```python
from build123d import *

# Parameters (mm, degrees)
SLOTTED_BASE_PLATE_DEPTH = 14
REAR_UPRIGHT_BLOCK_DEPTH = 23
UPPER_STEP_BLOCK_DEPTH   = 9
TOP_BLOCK_DEPTH          = 9


with BuildPart() as part:
    # Slotted Base Plate Sketch → Slotted Base Plate (new body)
    with BuildSketch(Plane(origin=(0, 0, 0), x_dir=(1, 0, 0), z_dir=(0, 1, 0))):
        Polygon((-45.527413465, -5.526673775), (-45.527413465, -13.526673775), (-36.527413465, -13.526673775), (-36.527413465, 32.473326225), (-45.527413465, 32.473326225), (-45.527413465, 24.473326225), (-54.527413465, 24.473326225), (-54.527413465, -5.526673775), align=None)
        with BuildLine():
            ThreePointArc((5.472586535, 16.473326225), (-1.527413465, 9.473326225), (5.472586535, 2.473326225))
            Line((5.472586535, 2.473326225), (27.472586535, 2.473326225))
            Line((27.472586535, 2.473326225), (27.472586535, -8.526673775))
            Line((27.472586535, -8.526673775), (-10.527413465, -13.526673775))
            Line((-10.527413465, -13.526673775), (-36.527413465, -13.526673775))
            Line((-36.527413465, -13.526673775), (-36.527413465, 32.473326225))
            Line((-36.527413465, 32.473326225), (-10.527413465, 32.473326225))
            Line((-10.527413465, 32.473326225), (27.472586535, 27.473326225))
            Line((27.472586535, 27.473326225), (27.472586535, 16.473326225))
            Line((27.472586535, 16.473326225), (5.472586535, 16.473326225))
        make_face()
    extrude(amount=SLOTTED_BASE_PLATE_DEPTH)

    # Rear Upright Block Sketch → Rear Upright Block (add)
    with BuildSketch(Plane(origin=(0, 0, 0), x_dir=(1, 0, 0), z_dir=(0, 1, 0))):
        Polygon((-45.527413465, 32.473326225), (-36.527413465, 32.473326225), (-36.527413465, -13.526673775), (-45.527413465, -13.526673775), (-45.527413465, -5.526673775), (-54.527413465, -5.526673775), (-54.527413465, 24.473326225), (-45.527413465, 24.473326225), align=None)
    extrude(amount=REAR_UPRIGHT_BLOCK_DEPTH)

    # Upper Step Sketch → Upper Step Block (add)
    with BuildSketch(Plane(origin=(-36.527413465, 0, 0), x_dir=(0, 0, -1), z_dir=(1, 0, 0))):
        Polygon((-13.526673775, 23), (32.473326225, 23), (16.473326225, 32.368724422), (2.473326225, 32.368724422), align=None)
    extrude(amount=-UPPER_STEP_BLOCK_DEPTH)

    # Top Block Sketch → Top Block (add)
    with BuildSketch(Plane.ZY.offset(45.527413465)):
        Polygon((-24.473326225, 23), (-24.473326225, 27.684362211), (-16.473326225, 32.368724422), (-2.473326225, 32.368724422), (5.526673775, 27.684362211), (5.526673775, 23), align=None)
    extrude(amount=TOP_BLOCK_DEPTH)


solid = part.part
```
The listing builds one solid part. Answer for the finished solid, in the listing's coordinates (mm). A direction names the side the tool comes from. Give positions to 0.01 mm unless a question says otherwise; leave off trailing zeros. Order: outer loops, then holes, each group sorted by start corner. A loop starts at its lowest first (then second) coordinate and runs counter-clockwise, first axis right, second up. Notation, with made-up numbers: M 72.5,-14 L 77.5,-14 A12 ccw 77.5,0 Z; hole C 82,12 d3. An arc over 180 degrees is marked long. Put each result on its own line as item: value. Start each with the question number.
Item 1: The part is cut by section D-D, the plane y = 19.5. Determine the outline of the cut face in (x, z).
Item 2: The part is cut by section B-B, the plane x = 8. Determine the outline of the cut face in (y, z).
Item 3: The part is cut by section A-A, the plane y = 10. Determine the outline of the cut face in (x, z), and give its area (3 significant figures).
Item 4: The part is cut by section C-C, the plane z = -22.5. Determine the outline of the cut face in (x, y), and give its area (3 significant figures).
Item 5: Flat-ended cylindrical pins translate along their axes: P1, Ø2.5, axis at y = 16.5, z = 10.5, coming from the -X side; P2, Ø4, axis at x = 13.5, y = 6.5, coming from the +Z side; P3, Ø9, axis at y = 20, z = -27.5, coming from the -X side; P4, Ø7, axis at x = -51, y = 11.5, coming from the -Z side. Find the tip coordinate at first contact, or state that the pin passes through.
Item 6: Which of the six approach directions +Z, -Z, +X, -X, +Y, -Y give full straight-line access (tool end or side, diameter ignored) to faces 5 (the face through (-12, 14, -10)), 6 (the face through (-50, 14, -24.473)), 7 (the face through (-45.527, 14, 10))?
Item 7: For a pull along Z with two mould halves and no side action, classify faces 1 (the face through (16, 7, -2.473)), 2 (the face through (-43.4, 28.79, 3.64)), 3 (the face through (-45.527, 14, -28)), 4 (the face through (17, 7, -16.473)) as +Z half, -Z half, draft (parallel to the pull), parting line (faces both ways), or undercut.
Item 8: Find the intervals of material crossed by line 1 along X through (y, z) = (20, -26); line 2 along Y through (x, z) = (-12, -1); line 3 along Z through (x, y) = (24.5, 4), in increasing order.
Answer key:
1. outline: M -54.53,-24.47 L -45.53,-24.47 L -45.53,-32.47 L -36.53,-32.47 L -36.53,13.53 L -45.53,13.53 L -45.53,5.53 L -54.53,5.53 Z
2. outline: M 0,-30.04 L 14,-30.04 L 14,-16.47 L 0,-16.47 Z; M 0,-2.47 L 14,-2.47 L 14,11.09 L 0,11.09 Z
3. outline: M -54.53,-24.47 L -45.53,-24.47 L -45.53,-32.47 L -10.53,-32.47 L 27.47,-27.47 L 27.47,-16.47 L 5.47,-16.47 A7 cw 5.47,-2.47 L 27.47,-2.47 L 27.47,8.53 L -10.53,13.53 L -45.53,13.53 L -45.53,5.53 L -54.53,5.53 Z
3. area: 3,050 mm²
4. outline: M -54.53,0 L 27.47,0 L 27.47,14 L -36.53,14 L -36.53,28.84 L -54.53,28.84 Z
4. area: 1,420 mm²
5. P1: stops at x = -45.53
5. P2: stops at z = 10.63
5. P3: stops at x = -54.53
5. P4: stops at z = -24.47
6. face 5: +Z, -Z, +X, +Y
6. face 6: -Z, -X, +Y, -Y
6. face 7: +Z, -X, +Y, -Y
7. face 1: undercut
7. face 2: +Z half
7. face 3: draft
7. face 4: undercut
8. line 1: x = -45.53 to -36.53
8. line 2: y = 0 to 14
8. line 3: z = -27.86 to -16.47, -2.47 to 8.92
